Read the model definition and answer for the solid it produces. Units are mm, in the model's axes. Face numbers are marked on the shaded views. A direction names the side the tool comes from. Coordinates: 2 decimals unless noted, no trailing zeros. Loops run counter-clockwise (first coordinate to the right, second up) from the corner with the lowest first, then second, coordinate; pieces in that order, holes last. Notation, with made-up numbers: M 18.25,68 L 48.25,68 A8 ccw 48.25,80 Z; hole C 4,-36.5 d6. An arc over 180 degrees is marked long. One line per item, written item: value. Start each with the question number.
1. The part is cut by section B-B (x = 21). Write down the section's boundary in (y, z), then the cut area to 3 significant figures.
2. The part is cut by section A-A (y = 0). Write down the section's boundary in (x, z), then the cut area to 3 significant figures.
3. Consider probe 1 along Y at (x, z) = (14.5, 30); probe 2 along Z at (x, y) = (26, 6.5); probe 3 along Z at (x, y) = (-17, 4.5). Determine where each line is inside the solid, lowest interval first.
4. The part is cut by section D-D (x = 34.5). Write down the section's boundary in (y, z), then the cut area to 3 significant figures.
5. Flat-ended cylindrical pins translate along their axes: pin 1 (10 mm diameter, centred on x = 74, z = 24.5, fed in from -Y); pin 2 (8 mm diameter, centred on x = 33, y = 12.5, fed in from -Z); pin 3 (3 mm diameter, centred on x = 51, z = 15.5, fed in from -Y); pin 4 (3 mm diameter, centred on x = 31, y = -9.5, fed in from +Z). Find the tip coordinate at first contact, or state that the pin passes through.
6. For the marked faces 4, 5 and 6, determine the directions among +Z, -Z, +X, -X, +Y, -Y from which every point of the face is accessible in a straight line to the end or side of a thin tool.
7. The part is cut by section C-C (z = 23.5). Write down the section's boundary in (x, y), then the cut area to 3 significant figures.
8. Determine the mould class of the marked faces 1, 2 and 3 for opening direction Y: +Y half, -Y half, draft (parallel to the pull), parting line (faces both ways), or undercut.
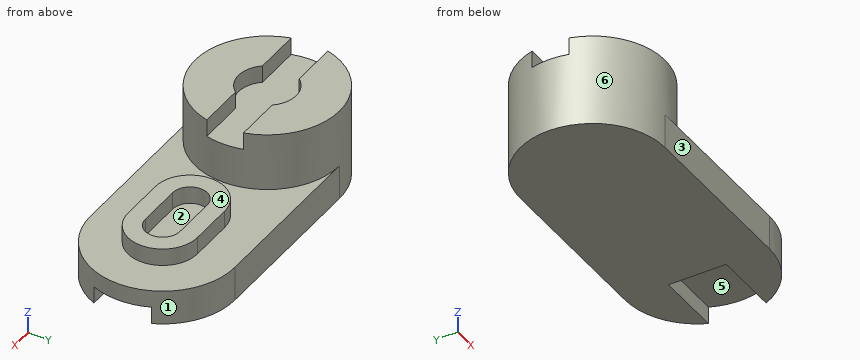
```python
from build123d import *

# Parameters (mm, degrees)
BASE_PLATE_DEPTH          = 12
HUB_BOSS_SKETCH_R         = 25
HUB_BOSS_DEPTH            = 20
HUB_START                 = -6
HUB_KEYHOLE_SLOT_SKETCH_R = 10
HUB_KEYHOLE_SLOT_DEPTH    = 6
SLOT_RIM_DEPTH            = 6
OBROUND_SLOT_DEPTH        = 95.201910809
OBROUND_SLOT_DEPTH_BACK   = 6


with BuildPart() as part:
    # Base Plate Sketch → Base Plate (new body)
    with BuildSketch(Plane.XY):
        with BuildLine():
            Line((0, 25), (60, 25))
            ThreePointArc((60, 25), (85, 0), (60, -25))
            Line((60, -25), (0, -25))
            ThreePointArc((0, -25), (-25, 0), (0, 25))
        make_face()
    extrude(amount=BASE_PLATE_DEPTH)

    # Hub Boss Sketch → Hub Boss (add)
    with BuildSketch(Plane.XY.offset(12)):
        with Locations(Location((0, 0, 0), (0, 0, 270))):
            Circle(HUB_BOSS_SKETCH_R)
    extrude(amount=HUB_BOSS_DEPTH)

    # Hub Keyhole Slot Sketch → Hub Keyhole Slot (cut)
    with BuildSketch(Plane.XY.offset(32).offset(HUB_START)):
        with BuildLine():
            ThreePointArc((-7.726954142, -6.347769662), (-10, 0), (-7.726954142, 6.347769662))
            Line((-7.726954142, 6.347769662), (-24.180691064, 6.347769662))
            ThreePointArc((-24.180691064, 6.347769662), (-25, 0), (-24.180691064, -6.347769662))
            Line((-24.180691064, -6.347769662), (-7.726954142, -6.347769662))
        make_face()
        Circle(HUB_KEYHOLE_SLOT_SKETCH_R)
        with BuildLine():
            Line((24.180691064, 6.347769662), (7.726954142, 6.347769662))
            ThreePointArc((7.726954142, 6.347769662), (9.414604119, 3.371235573), (10, 0))
            ThreePointArc((10, 0), (9.414604119, -3.371235573), (7.726954142, -6.347769662))
            Line((7.726954142, -6.347769662), (24.180691064, -6.347769662))
            ThreePointArc((24.180691064, -6.347769662), (24.794326736, -3.200212759), (25, 0))
            ThreePointArc((25, 0), (24.794326736, 3.200212759), (24.180691064, 6.347769662))
        make_face()
    extrude(amount=HUB_KEYHOLE_SLOT_DEPTH, mode=Mode.SUBTRACT)

    # Slot Rim Sketch → Slot Rim (add)
    with BuildSketch(Plane.XY.offset(12)):
        with BuildLine():
            Line((44.323016702, 12), (60, 12))
            ThreePointArc((60, 12), (72, 0), (60, -12))
            Line((60, -12), (44.323016702, -12))
            ThreePointArc((44.323016702, -12), (32.323016702, 0), (44.323016702, 12))
        make_face()
        with BuildLine():
            Line((44.323016702, 6), (60, 6))
            ThreePointArc((60, 6), (66, 0), (60, -6))
            Line((60, -6), (44.323016702, -6))
            ThreePointArc((44.323016702, -6), (38.323016702, 0), (44.323016702, 6))
        make_face(mode=Mode.SUBTRACT)
    extrude(amount=SLOT_RIM_DEPTH)

    # Obround Slot Sketch → Obround Slot (cut, two sides: drawn at the far end of the back side and taken through both)
    with BuildSketch(Plane(origin=(0, 0, 0), x_dir=(-1, 0, 0), z_dir=(0, 0, -1)).offset(-OBROUND_SLOT_DEPTH_BACK)):
        with BuildLine():
            ThreePointArc((-82.912878475, 10), (-85, 0), (-82.912878475, -10))
            Line((-82.912878475, -10), (-60, -10))
            Line((-60, -10), (-60, 10))
            Line((-60, 10), (-82.912878475, 10))
        make_face()
    extrude(amount=OBROUND_SLOT_DEPTH + OBROUND_SLOT_DEPTH_BACK, mode=Mode.SUBTRACT)


solid = part.part
```
Answer block:
1. outline: M -25,0 L 25,0 L 25,12 L 13.56,12 L 13.56,32 L 6.35,32 L 6.35,26 L -6.35,26 L -6.35,32 L -13.56,32 L -13.56,12 L -25,12 Z
1. area: 1,070 mm2
2. outline: M -25,0 L 60,0 L 60,6 L 85,6 L 85,12 L 72,12 L 72,18 L 66,18 L 66,12 L 38.32,12 L 38.32,18 L 32.32,18 L 32.32,12 L 25,12 L 25,26 L -25,26 Z
2. area: 1,940 mm2
3. probe 1: y = -20.37 to -6.35, 6.35 to 20.37
3. probe 2: z = 0 to 12
3. probe 3: z = 0 to 26
4. outline: M -25,0 L 25,0 L 25,12 L 6.89,12 L 6.89,18 L -6.89,18 L -6.89,12 L -25,12 Z
4. area: 683 mm2
5. pin 1: passes through
5. pin 2: stops at z = 0
5. pin 3: stops at y = -12
5. pin 4: stops at z = 12
6. face 4: +Z, +X, +Y, -Y
6. face 5: -Z, +X
6. face 6: +Z
7. outline: C 0,0 d50
7. area: 1,960 mm2
8. face 1: parting line
8. face 2: undercut
8. face 3: -Y half
